Design review of the part built by this model. Coordinates are the model's own, in mm. Face numbers are marked on the shaded views. Give positions to 0.01 mm unless a question says otherwise; leave off trailing zeros. Order: outer loops, then holes, each group sorted by start corner. A loop starts at its lowest first (then second) coordinate and runs counter-clockwise, first axis right, second up. Notation, with made-up numbers: (60.25, 9) -> (99.25, 9) arc R17 cw to (99.25, 19) -> close; hole circle Ø9 at (50.25, -35). An arc over 180 degrees is marked (long way). Answer in a Markdown table with one row per item. Add a question column.
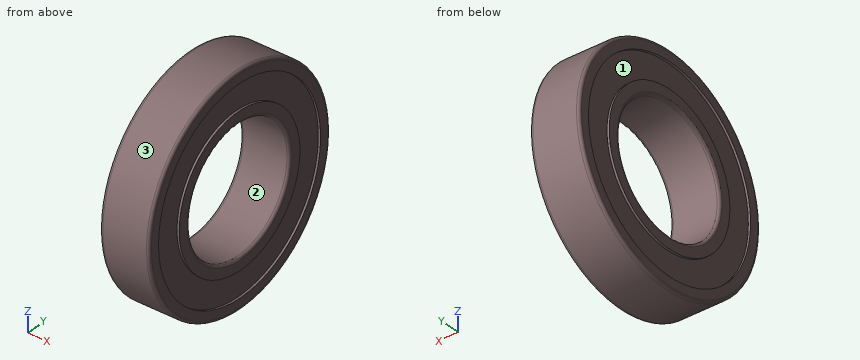
```python
from build123d import *

# Parameters (mm, degrees)
FILLET1_R = 1.1
FILLET2_R = 1.1


with BuildPart() as part:
    # Sketch1 → Revolve1 (revolve)
    with BuildSketch(Plane.XY, mode=Mode.PRIVATE) as revolve1_sk:
        Polygon((0, 25), (20, 25), (20, 30.05), (19.08, 30.05), (19.08, 40.35), (20, 40.35), (20, 45), (0, 45), (0, 40.35), (0.92, 40.35), (0.92, 30.05), (0, 30.05), align=None)
    revolve(revolve1_sk.sketch.rotate(Axis((0, 0, 0), (1, 0, 0)), 180), axis=Axis((0, 0, 0), (1, 0, 0)))

    # Fillet1
    fillet1_edges = [part.edges().sort_by_distance(p)[0] for p in [
        (0, 45, 0),
        (20, 45, 0),
    ]]
    fillet(fillet1_edges, radius=FILLET1_R)

    # Fillet2
    fillet2_edges = [part.edges().sort_by_distance(p)[0] for p in [
        (20, 25, 0),
        (0, 25, 0),
    ]]
    fillet(fillet2_edges, radius=FILLET2_R)


solid = part.part
```
1) For L1, parallel to Y at x = 3.25, z = 1; L2, parallel to Z at x = 14.75, y = 0; L3, parallel to Z at x = 19.75, y = 0, list the stretches that pass through material, from the lowest coordinate up.
2) Add section C-C, the plane x = 5.5. Write out the cut boundary in (y, z).
3) Clearance check with flat-ended pins moving along their axes: P1, Ø1, axis at x = 16.5, z = 2.5, coming from the -Y side; P2, Ø6, axis at x = 11.5, z = -28.5, coming from the -Y side; P3, Ø10, axis at x = 8.5, y = 31.5, coming from the +Z side. State where each tip first meets the part, or that it passes through.
4) Mouldability with a two-part tool opening along Y and no side actions: class the marked faces 1, 2 and 3 as +Y half, -Y half, draft (parallel to the pull), parting line (faces both ways), or undercut.
Verdict:
| question | item | result |
|---|---|---|
| 1 | L1 | y = -44.99 to -24.98, 24.98 to 44.99 |
| 1 | L2 | z = -45 to -25, 25 to 45 |
| 1 | L3 | z = -44.6 to -40.35, -30.05 to -25.4, 25.4 to 30.05, 40.35 to 44.6 |
| 2 | outline | circle Ø90 at (0, 0); hole circle Ø50 at (0, 0) |
| 3 | P1 | stops at y = -44.96 |
| 3 | P2 | stops at y = -37.08 |
| 3 | P3 | stops at z = 36.37 |
| 4 | face 1 | undercut |
| 4 | face 2 | undercut |
| 4 | face 3 | parting line |
